from build123d import *

# Parameters (mm, degrees)
BASE_BLOCK_95_DEPTH      = 47.5
UPRIGHT_BLOCK_40_DEPTH   = 40
RELIEF_GROOVE_SKETCH_W   = 3
RELIEF_GROOVE_SKETCH_H   = 10
RELIEF_GROOVE_3X10_DEPTH = 144.227092409
UPRIGHT_FILLET_R2_R      = 2
TOP_SLOT_SKETCH_W        = 71
TOP_SLOT_SKETCH_H        = 10
TOP_SLOT_10_WIDE_DEPTH   = 12
V_NOTCH_DEPTH            = 151.499169433
RAISED_PAD_3MM_DEPTH     = 3
PAD_FILLET_R2_R          = 2
PAD_U_SLOT_12_WIDE_DEPTH = 3


with BuildPart() as part:
    # Base Profile Sketch → Base Block 95 (new, symmetric)
    with BuildSketch(Plane(origin=(0, 0, 0), x_dir=(0, 0, -1), z_dir=(1, 0, 0))):
        Polygon((0, 0), (50, 0), (50, 7), (70, 7), (70, 0), (80, 0), (80, 25), (0, 25), align=None)
    extrude(amount=BASE_BLOCK_95_DEPTH, both=True)

    # Upright Profile Sketch → Upright Block 40 (add)
    with BuildSketch(Plane.XY):
        Polygon((-47.5, 25), (-47.5, 85), (10.5, 85), (35.5, 60), (35.5, 25), align=None)
    extrude(amount=-UPRIGHT_BLOCK_40_DEPTH)

    # Relief Groove Sketch → Relief Groove 3x10 (cut, through all)
    with BuildSketch(Plane(origin=(35.5, 0, 0), x_dir=(0, 0, -1), z_dir=(1, 0, 0))):
        with Locations((38.5, 30)):
            Rectangle(RELIEF_GROOVE_SKETCH_W, RELIEF_GROOVE_SKETCH_H)
    extrude(amount=-RELIEF_GROOVE_3X10_DEPTH, mode=Mode.SUBTRACT)

    # Upright Fillet R2
    upright_fillet_r2_edges = [part.edges().sort_by_distance(p)[0] for p in [
        (35.5, 25, -18.5),
        (-6, 25, -37),
        (-6, 35, -37),
        (35.5, 35, -38.5),
        (35.5, 30, -37),
    ]]
    fillet(upright_fillet_r2_edges, radius=UPRIGHT_FILLET_R2_R)

    # Top Slot Sketch → Top Slot 10 Wide (cut)
    with BuildSketch(Plane(origin=(0, 85, 0), x_dir=(1, 0, 0), z_dir=(0, 1, 0))):
        with Locations((-12, 20)):
            Rectangle(TOP_SLOT_SKETCH_W, TOP_SLOT_SKETCH_H)
    extrude(amount=-TOP_SLOT_10_WIDE_DEPTH, mode=Mode.SUBTRACT)

    # V Notch Sketch → V Notch (cut, through all)
    with BuildSketch(Plane.ZY.offset(47.5)):
        Polygon((0, 60), (0, 85), (-10, 85), align=None)
    extrude(amount=-V_NOTCH_DEPTH, mode=Mode.SUBTRACT)

    # Raised Pad Sketch → Raised Pad 3mm (add)
    with BuildSketch(Plane(origin=(0, 25, 0), x_dir=(1, 0, 0), z_dir=(0, 1, 0))):
        with BuildLine():
            Line((-22.5, 72), (22.5, 72))
            ThreePointArc((22.5, 72), (34.5, 60), (22.5, 48))
            Line((22.5, 48), (-22.5, 48))
            ThreePointArc((-22.5, 48), (-34.5, 60), (-22.5, 72))
        make_face()
    extrude(amount=RAISED_PAD_3MM_DEPTH)

    # Pad Fillet R2
    pad_fillet_r2_edges = [part.edges().sort_by_distance(p)[0] for p in [
        (-34.5, 25, -60),
        (0, 25, -48),
        (34.5, 25, -60),
        (0, 25, -72),
    ]]
    fillet(pad_fillet_r2_edges, radius=PAD_FILLET_R2_R)

    # Pad Slot Sketch → Pad U-Slot 12 Wide (cut)
    with BuildSketch(Plane(origin=(0, 28, 0), x_dir=(1, 0, 0), z_dir=(0, 1, 0))):
        with BuildLine():
            Line((-22.5, 66), (22.5, 66))
            ThreePointArc((22.5, 66), (28.5, 60), (22.5, 54))
            Line((22.5, 54), (-22.5, 54))
            ThreePointArc((-22.5, 54), (-28.5, 60), (-22.5, 66))
        make_face()
    extrude(amount=-PAD_U_SLOT_12_WIDE_DEPTH, mode=Mode.SUBTRACT)


solid = part.part
The model under review builds one solid part; all positions refer to its coordinate system, in mm. A direction names the side the tool comes from. Round coordinates to 2 decimals unless told otherwise and drop trailing zeros. Loops run counter-clockwise (first coordinate to the right, second up) from the corner with the lowest first, then second, coordinate; pieces in that order, holes last. Notation, with made-up numbers: (68, -28.5) -> (91, -28.5) arc R31 cw to (91, -2.5) -> close; hole circle Ø5 at (27.25, -31.75). An arc over 180 degrees is marked (long way). Return JSON: item names as keys, results as strings.
(1) Add section D-D on z = -60. Write out the cut boundary in (x, y), plus the area to 3 significant figures.
Solved:
{"outline": "(-47.5, 7) -> (47.5, 7) -> (47.5, 25) -> (36.5, 25) arc R2 cw to (34.5, 27) -> (34.5, 28) -> (28.5, 28) -> (28.5, 25) -> (-28.5, 25) -> (-28.5, 28) -> (-34.5, 28) -> (-34.5, 27) arc R2 cw to (-36.5, 25) -> (-47.5, 25) -> close", "area": "1,750 mm2"}
(2) Add section B-B on z = -33. Write out the cut boundary in (x, y), plus the area to 3 significant figures.
Solved:
{"outline": "(-47.5, 0) -> (47.5, 0) -> (47.5, 25) -> (37.5, 25) arc R2 cw to (35.5, 27) -> (35.5, 60) -> (10.5, 85) -> (-47.5, 85) -> close", "area": "7,040 mm2"}
(3) For faces 1 (the flat face through (0, 27, -54)), 2 (the flat face through (1, 3, -50)), 3 (the cylindrical face through (34.497, 27.493, -60.264)), list the 3-axis set-ups (+Z, -Z, +X, -X, +Y, -Y) from which the entire face can be reached by the end or side of a thin tool; tool diameter is ignored.
Solved:
{"face 1": "+Y", "face 2": "+X, -X, -Y", "face 3": "+X, +Y"}
(4) Add section A-A on y = 74.5. Write out the cut boundary in (x, z).
Solved:
{"outline": "(-47.5, -40) -> (21, -40) -> (21, -25) -> (-47.5, -25) -> close; (-47.5, -15) -> (21, -15) -> (21, -5.8) -> (-47.5, -5.8) -> close"}
(5) For line 1 (Y direction, x = 29.5, z = -61.5); line 2 (Y direction, x = 37, z = -56.5); line 3 (Z direction, x = 5, y = 73.5), list the stretches that pass through material, from the lowest coordinate up.
Solved:
{"line 1": "7 to 28", "line 2": "7 to 25", "line 3": "-40 to -25, -15 to -5.4"}
(6) The part is to be moulded in two halves that separate along X. For faces 4 (the flat face through (35.5, 44, -20)), 5 (the flat face through (-19, 85, -12)), 6 (the cylindrical face through (-28.5, 26.5, -59.9)), say which applies: released by +X, released by -X, zero draft, split by the parting line, or undercut.
Solved:
{"face 4": "released by +X", "face 5": "zero draft", "face 6": "undercut"}
(7) For pin 1 (6 mm diameter, centred on x = -11.5, z = -59, fed in from +Y); pin 2 (4 mm diameter, centred on y = 27.5, z = -20, fed in from +X); pin 3 (6 mm diameter, centred on x = 2.5, y = 76.5, fed in from +Z), all flat-tipped, find the tip position at first contact; note any pin that passes through.
Solved:
{"pin 1": "y = 25", "pin 2": "x = 36.18", "pin 3": "z = -5.4"}
